Geometry: see drawing. Coordinates: mm, zero at the bounding-box minimum. Coordinates: 2 decimals unless noted, no trailing zeros. Write each loop counter-clockwise with the first axis right and the second up, starting at its lowest first coordinate (ties: lowest second). Pieces come first, ordered by that corner, then holes.
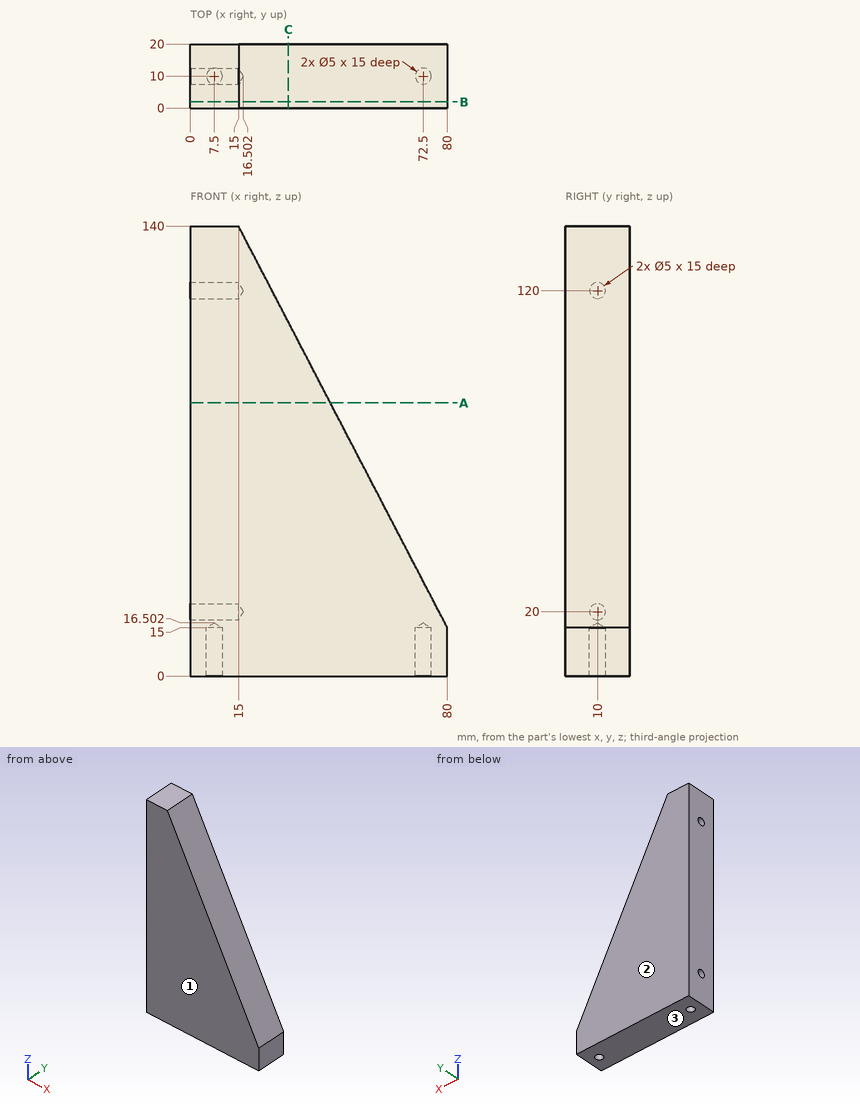
Item 1: Section A-A, the plane z = 85. Output: boundary loops of the cut face in (x, y).
Derived:
outline: (0, 0) - (43.6, 0) - (43.6, 20) - (0, 20) - close
Item 2: Pull-direction query (Y, two-part tool) for the marked faces 1, 2 and 3; classes: released by +Y, released by -Y, zero draft, split by the parting line, or undercut.
Derived:
face 1: released by -Y
face 2: released by +Y
face 3: zero draft
Item 3: Section B-B, the plane y = 2. Output: boundary loops of the cut face in (x, z), plus the area to 3 significant figures.
Derived:
outline: (0, 0) - (80, 0) - (80, 15) - (15, 140) - (0, 140) - close
area: 7,140 mm2
Item 4: Pin query (flat end, axial travel): pin 1 (1.5 mm diameter, centred on y = 12, z = 37.5, fed in from -X); pin 2 (3 mm diameter, centred on x = 72.5, y = 10, fed in from -Z); pin 3 (1.5 mm diameter, centred on x = 46.5, y = 17.5, fed in from +Z) (1 decimal); pin 4 (1.5 mm diameter, centred on x = 53, y = 11, fed in from +Z) (1 decimal). Return the tip coordinate at first contact, or that it passes through.
Derived:
pin 1: stops at x = 0
pin 2: stops at z = 15.6
pin 3: stops at z = 80.9
pin 4: stops at z = 68.4
Item 5: Section C-C, the plane x = 30.5. Output: boundary loops of the cut face in (y, z).
Derived:
outline: (0, 0) - (20, 0) - (20, 110.19) - (0, 110.19) - close
Item 6: Material intervals for probe 1 along Z at (x, y) = (4, 10); probe 2 along X at (y, z) = (10, 3.5); probe 3 along Y at (x, z) = (4, 120), sorted ascending.
Derived:
probe 1: z = 0 to 17.5, 22.5 to 117.5, 122.5 to 140
probe 2: x = 0 to 5, 10 to 70, 75 to 80
probe 3: y = 0 to 7.5, 12.5 to 20
